```python
from build123d import *

# Parameters (mm, degrees)
SKETCH_1_R         = 52.5
SKETCH_1_R_2       = 47.5
EXTRUDE_1_DEPTH    = 5
CHAMFER_1_SIZE     = 0.5
HOLE_WIZARD_M6_1_D = 5


with BuildPart() as part:
    # 草图1 → 凸台-拉伸1 (new, symmetric)
    with BuildSketch(Plane(origin=(0, 0, 0), x_dir=(0, 0, -1), z_dir=(1, 0, 0))):
        Circle(SKETCH_1_R)
        Circle(SKETCH_1_R_2, mode=Mode.SUBTRACT)
    extrude(amount=EXTRUDE_1_DEPTH, both=True)

    # 倒角1
    chamfer_1_edges = [part.edges().sort_by_distance(p)[0] for p in [
        (-5, 0, 52.5),
        (5, 0, 52.5),
        (-5, 0, 47.5),
        (5, 0, 47.5),
    ]]
    chamfer(chamfer_1_edges, length=CHAMFER_1_SIZE)

    # M6 螺纹孔1 (through all)
    with Locations(Plane(origin=(0, 52.5, 0), x_dir=(1, 0, 0), z_dir=(0, 1, 0))):
        with Locations((0, 0)):
            Hole(HOLE_WIZARD_M6_1_D / 2)


solid = part.part
```
CAD build for the part. Positions are in the model's coordinates, mm. Round coordinates to 2 decimals unless told otherwise and drop trailing zeros. Loops run counter-clockwise (first coordinate to the right, second up) from the corner with the lowest first, then second, coordinate; pieces in that order, holes last. Notation, with made-up numbers: (14.25, 46) - (38.25, 46) arc R17 ccw to (38.25, 68) - close; hole circle Ø3 at (-37, 9.25). An arc over 180 degrees is marked (long way). Return JSON: item names as keys, results as strings. Group by question number.
Q1. Drill centre lines: line 1 along Y through (x, z) = (0, 38.5); line 2 along Z through (x, y) = (1.75, -41.5); line 3 along Y through (x, z) = (-3.75, -6). Where is each one in solid material? Low to high. Write a range as [from, to].
Q2. Band-saw the part on A-A on y = 0. Give the cut face in (x, z), plus the area to 3 significant figures.
Q3. Band-saw the part on B-B on z = 0. Give the cut face in (x, y).
Q4. Flat gauge pins, fed straight in: pin 1 Ø1 at (x, z) = (3, 8) entering from -Y; pin 2 Ø3 at (x, y) = (-3.5, 3) entering from -Z; pin 3 Ø4 at (x, y) = (1, 9) entering from +Z. Where does each tip first touch, or does it go through?
Q5. Two-plate mould, pull along Y, no slides. Class faces 1 (the face through (0.54, -50, 2.44)), 2 (the face through (0.063, 15.77, -50.076)), 3 (the face through (-0.06, -46.37, 10.3)): +Y half, -Y half, draft (parallel to the pull), parting line (faces both ways), or undercut.
Solutions:
{
 "1": {"line 1": "y = [-35.69, -27.82], [27.82, 35.69]", "line 2": "z = [-32.16, -23.11], [23.11, 32.16]", "line 3": "y = [-52.16, -47.12], [47.12, 52.16]"},
 "2": {"outline": "(-5, -52) - (-4.5, -52.5) - (4.5, -52.5) - (5, -52) - (5, -48) - (4.5, -47.5) - (-4.5, -47.5) - (-5, -48) - close; (-5, 48) - (-4.5, 47.5) - (4.5, 47.5) - (5, 48) - (5, 52) - (4.5, 52.5) - (-4.5, 52.5) - (-5, 52) - close", "area": "99.0 mm^2"},
 "3": {"outline": "(-5, -52) - (-4.5, -52.5) - (-2.5, -52.5) - (-2.5, -47.5) - (-4.5, -47.5) - (-5, -48) - close; (-5, 48) - (-4.5, 47.5) - (-2.5, 47.5) - (-2.5, 52.5) - (-4.5, 52.5) - (-5, 52) - close; (2.5, -52.5) - (4.5, -52.5) - (5, -52) - (5, -48) - (4.5, -47.5) - (2.5, -47.5) - close; (2.5, 47.5) - (4.5, 47.5) - (5, 48) - (5, 52) - (4.5, 52.5) - (2.5, 52.5) - close"},
 "4": {"pin 1": "stops at y = -51.96", "pin 2": "stops at z = -52.48", "pin 3": "stops at z = 52.03"},
 "5": {"face 1": "draft", "face 2": "parting line", "face 3": "undercut"}
}
